Read the model definition and answer for the solid it produces. Units are mm, in the model's axes. Coordinates: 2 decimals unless noted, no trailing zeros. Loops run counter-clockwise (first coordinate to the right, second up) from the corner with the lowest first, then second, coordinate; pieces in that order, holes last. Notation, with made-up numbers: (-17.5, 39) -> (9.5, 39) arc R19 ccw to (9.5, 76) -> close; hole circle Ø3 at (69.25, 33.25). An arc over 180 degrees is marked (long way). Answer as CSV lines item,"result".
```python
from build123d import *

# Parameters (mm, degrees)
SKETCH1_W           = 15
SKETCH1_H           = 24
BOSS_EXTRUDE1_DEPTH = 1
FILLET1_R           = 2


with BuildPart() as part:
    # Sketch1 → Boss-Extrude1 (new body)
    with BuildSketch(Plane.XY):
        Rectangle(SKETCH1_W, SKETCH1_H)
        with BuildLine():
            Line((-4, 8.75), (4, 8.75))
            ThreePointArc((4, 8.75), (5.75, 7), (4, 5.25))
            Line((4, 5.25), (-4, 5.25))
            ThreePointArc((-4, 5.25), (-5.75, 7), (-4, 8.75))
        make_face(mode=Mode.SUBTRACT)
    extrude(amount=BOSS_EXTRUDE1_DEPTH)

    # Fillet1
    fillet1_edges = [part.edges().sort_by_distance(p)[0] for p in [
        (7.5, -12, 0.5),
        (-7.5, -12, 0.5),
        (-7.5, 12, 0.5),
        (7.5, 12, 0.5),
    ]]
    fillet(fillet1_edges, radius=FILLET1_R)


solid = part.part
```
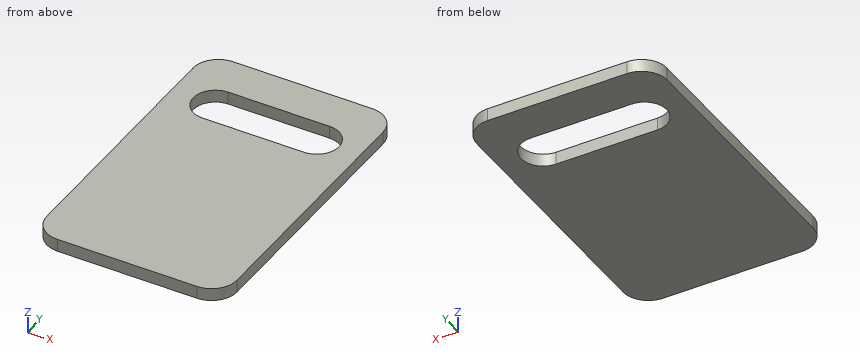
Q1. A cutting plane is placed at C-C, the plane z = 0.4. Write down the section's boundary in (x, y), and give its area (3 significant figures).
Results:
outline,"(-7.5, -10) arc R2 ccw to (-5.5, -12) -> (5.5, -12) arc R2 ccw to (7.5, -10) -> (7.5, 10) arc R2 ccw to (5.5, 12) -> (-5.5, 12) arc R2 ccw to (-7.5, 10) -> close; hole (-4, 5.25) -> (4, 5.25) arc R1.75 ccw to (4, 8.75) -> (-4, 8.75) arc R1.75 ccw to start"
area,"319 mm²"
Q2. A cutting plane is placed at A-A, the plane y = 7. Write down the section's boundary in (x, z).
Results:
outline,"(-7.5, 0) -> (-5.75, 0) -> (-5.75, 1) -> (-7.5, 1) -> close; (5.75, 0) -> (7.5, 0) -> (7.5, 1) -> (5.75, 1) -> close"
Q3. A cutting plane is placed at D-D, the plane x = 6.5. Write down the section's boundary in (y, z).
Results:
outline,"(-11.73, 0) -> (11.73, 0) -> (11.73, 1) -> (-11.73, 1) -> close"
Q4. Find the intervals of material crossed by probe 1 along Y at (x, z) = (1.75, 0.25); probe 2 along Y at (x, z) = (-4.75, 0.35); probe 3 along X at (y, z) = (5.75, 0.45), in increasing order. Write a range as [from, to].
Results:
probe 1,"y = [-12, 5.25], [8.75, 12]"
probe 2,"y = [-12, 5.42], [8.58, 12]"
probe 3,"x = [-7.5, -5.22], [5.22, 7.5]"
Q5. A cutting plane is placed at B-B, the plane x = 0.5. Write down the section's boundary in (y, z), and give its area (3 significant figures).
Results:
outline,"(-12, 0) -> (5.25, 0) -> (5.25, 1) -> (-12, 1) -> close; (8.75, 0) -> (12, 0) -> (12, 1) -> (8.75, 1) -> close"
area,"20.5 mm²"
